```python
from build123d import *

# Parameters (mm, degrees)
SKETCH_1_W                = 65
SKETCH_1_H                = 370
EXTRUDE_1_DEPTH           = 12
HOLE_WIZARD_M8_1_D        = 6.8
HOLE_WIZARD_1_D           = 4.5
HOLE_WIZARD_1_CBORE_D     = 8
HOLE_WIZARD_1_CBORE_DEPTH = 4.6
CHAMFER_1_SIZE            = 2
PATTERN_LINEAR_1_COUNT    = 2
PATTERN_LINEAR_1_PITCH    = 10


with BuildPart() as part:
    # 草图1 → 凸台-拉伸1 (new body)
    with BuildSketch(Plane(origin=(0, 0, 0), x_dir=(1, 0, 0), z_dir=(0, 1, 0))):
        Rectangle(SKETCH_1_W, SKETCH_1_H)
    extrude(amount=EXTRUDE_1_DEPTH)

    # M8 螺纹孔1 (through all)
    with Locations(Plane(origin=(0, 12, 0), x_dir=(1, 0, 0), z_dir=(0, 1, 0))):
        with Locations((25, -174), (25, -116), (25, -58), (25, 0), (25, 58), (25, 116), (25, 174)):
            Hole(HOLE_WIZARD_M8_1_D / 2)

    # 打孔尺寸(%根据)内六角圆柱头螺钉的类型1 (through all)
    with Locations(Plane(origin=(0, 0, 0), x_dir=(-1, 0, 0), z_dir=(0, -1, 0))):
        with Locations((27.5, -180), (27.5, -60), (27.5, 60), (27.5, 180)):
            hole_wizard_1 = CounterBoreHole(HOLE_WIZARD_1_D / 2, HOLE_WIZARD_1_CBORE_D / 2, HOLE_WIZARD_1_CBORE_DEPTH)

    # 倒角1
    chamfer_1_edges = [part.edges().sort_by_distance(p)[0] for p in [
        (32.5, 6, 185),
        (-32.5, 6, 185),
        (-32.5, 6, -185),
        (32.5, 6, -185),
    ]]
    chamfer(chamfer_1_edges, length=CHAMFER_1_SIZE)

    # 阵列(线性)1: 打孔尺寸(%根据)内六角圆柱头螺钉的类型1 ×2
    with Locations(*[(i * PATTERN_LINEAR_1_PITCH, 0, 0) for i in range(1, PATTERN_LINEAR_1_COUNT)]):
        add(hole_wizard_1, mode=Mode.SUBTRACT)


solid = part.part
```
Check sheet for the modelled part. Datum: model origin and axes. Units: mm. A direction names the side the tool comes from. Give positions to 0.01 mm unless a question says otherwise; leave off trailing zeros. Order: outer loops, then holes, each group sorted by start corner. A loop starts at its lowest first (then second) coordinate and runs counter-clockwise, first axis right, second up. Notation, with made-up numbers: M 12.25,42 L 71.25,42 A26 cw 71.25,70 Z; hole C -2,81.25 d4. An arc over 180 degrees is marked long. Answer in a Markdown table with one row per item. Add a question column.
Q1. Release check for a two-part mould opening along X. For faces 1 (the flat face through (-29, 4.6, -178)), 2 (the flat face through (32.5, 6, 3)), 3 (the flat face through (0, 0, -3)), 4 (the cylindrical face through (21.757, 5.916, 114.979)) record: released by +X, released by -X, zero draft, split by the parting line, or undercut.
Q2. Sectioned sample at B-B, the plane z = 116. Record the boundary of the cut face in (x, y), and give its area (3 significant figures).
Q3. Access from +Z, -Z, +X, -X, +Y, -Y to the whole of each face (thin tool, end or side, straight path). Record for faces 5 (the cylindrical face through (-26.633, 2.268, -56.095)), 6 (the cylindrical face through (23.172, 5.916, -118.867)).
Q4. Sectioned sample at A-A, the plane y = 2.5. Count the separate pieces of the cut face and the enclosed holes in it, and give its area (3 significant figures).
Q5. Thickness scan on L1, parallel to X at y = 7, z = -180; L2, parallel to X at y = 3.1, z = 180; L3, parallel to Z at x = -27.5, y = 7.5. Record the ranges inside material, lowest first.
Q6. Gauge pin test, flat ends, axial feed: pin 1 Ø2.5 at (x, z) = (-19, -58.5) entering from -Y; pin 2 Ø6 at (x, z) = (25, -58) entering from -Y. Record the tip position at first contact, or that the pin passes through.
Verdict:
| question | item | result |
|---|---|---|
| 1 | face 1 | undercut |
| 1 | face 2 | released by +X |
| 1 | face 3 | zero draft |
| 1 | face 4 | undercut |
| 2 | outline | M -32.5,0 L 21.6,0 L 21.6,12 L -32.5,12 Z; M 28.4,0 L 32.5,0 L 32.5,12 L 28.4,12 Z |
| 2 | area | 698 mm² |
| 3 | face 5 | -Y |
| 3 | face 6 | +Y, -Y |
| 4 | separate pieces | 1 |
| 4 | enclosed holes | 15 |
| 4 | area | 23,400 mm² |
| 5 | L1 | -32.5 to -29.75, -25.25 to -19.75, -15.25 to 32.5 |
| 5 | L2 | -32.5 to -31.5, -23.5 to -21.5, -13.5 to 32.5 |
| 5 | L3 | -185 to -182.25, -177.75 to -62.25, -57.75 to 57.75, 62.25 to 177.75, 182.25 to 185 |
| 6 | pin 1 | y = 4.6 |
| 6 | pin 2 | through |
